The model under review builds one solid part; all positions refer to its coordinate system, in mm. A direction names the side the tool comes from. Round coordinates to 2 decimals unless told otherwise and drop trailing zeros. Order: outer loops, then holes, each group sorted by start corner. A loop starts at its lowest first (then second) coordinate and runs counter-clockwise, first axis right, second up. Notation, with made-up numbers: M 72,26 L 89,26 A21 cw 89,30 Z; hole C -7.75,1 d9. An arc over 180 degrees is marked long. Answer as a JSON object with one key per item and string values. Group by question number.
1. To check wall thickness, follow probe 1 along Z at (x, y) = (-0.5, 9.25); probe 2 along X at (y, z) = (-3.25, 2); probe 3 along X at (y, z) = (-0.5, -55). State the ranges of each line that lie inside material, in increasing order. Write a range as [from, to].
2. Clearance check with flat-ended pins moving along their axes: P1, Ø2, axis at x = -8, z = 170.5, coming from the +Y side; P2, Ø1, axis at y = -7, z = 224.5, coming from the -X side; P3, Ø3, axis at y = 5.5, z = -22.5, coming from the +X side. State where each tip first meets the part, or that it passes through.
3. Machinability: for faces 1 (the face through (4.032, -6.324, -37.264)), 2 (the face through (-5.78, -7.54, 254.46)), 3 (the face through (-1.63, -7.32, 336.24)), which of the approach directions +Z, -Z, +X, -X, +Y, -Y give a long, thin tool a straight path to every point of the face, cutting with its end or side? Answer none if there is none.
4. Add section B-B on z = 219. State the section outline as (x, y) points.
5. Add section A-A on y = 0. State the section outline as (x, z) points, and give its area (3 significant figures).
6. Mouldability with a two-part tool opening along Z and no side actions: class faces 4 (the face through (-9, -4, 253.9)), 5 (the face through (0, 0, -74)), 6 (the face through (-9, -4, 255)), 7 (the face through (-7, 4, 300)) as released by +Z, released by -Z, zero draft, split by the parting line, or undercut.
```python
from build123d import *

# Parameters (mm, degrees)
SKETCH_1_R          = 10
EXTRUDE_1_DEPTH     = 300
SKETCH_2_R          = 6
EXTRUDE_2_DEPTH     = 74
EXTRUDE_START       = 74
SKETCH_3_R          = 6
EXTRUDE_3_DEPTH     = 74
SKETCH_4_R          = 7.5
EXTRUDE_4_DEPTH     = 74
SKETCH_5_R          = 7.5
EXTRUDE_5_DEPTH     = 74
CUT_EXTRUDE_1_DEPTH = 3
CHAMFER_1_SIZE      = 0.5
SKETCH_8_R          = 12.5
SKETCH_8_R_2        = 9.5
CUT_EXTRUDE_2_DEPTH = 1.1


with BuildPart() as part:
    # 草图1 → 凸台-拉伸1 (new body)
    with BuildSketch(Plane.XY):
        with Locations(Location((0, 0, 0), (0, 0, 90))):
            Circle(SKETCH_1_R)
    extrude(amount=EXTRUDE_1_DEPTH)

    # 草图2 → 凸台-拉伸2 (add)
    with BuildSketch(Plane(origin=(0, 0, 0), x_dir=(-1, 0, 0), z_dir=(0, 0, -1))):
        Circle(SKETCH_2_R)
    extrude(amount=EXTRUDE_2_DEPTH)

    # 草图3 → 凸台-拉伸3 (add)
    with BuildSketch(Plane.XY.offset(300).offset(EXTRUDE_START)):
        Circle(SKETCH_3_R)
    extrude(amount=-EXTRUDE_3_DEPTH)

    # 草图4 → 凸台-拉伸4 (add)
    with BuildSketch(Plane.XY.offset(300)):
        Circle(SKETCH_4_R)
    extrude(amount=EXTRUDE_4_DEPTH)

    # 草图5 → 凸台-拉伸5 (add)
    with BuildSketch(Plane(origin=(0, 0, 0), x_dir=(-1, 0, 0), z_dir=(0, 0, -1)).offset(EXTRUDE_START)):
        with Locations(Location((0, 0, 0), (0, 0, 180))):
            Circle(SKETCH_5_R)
    extrude(amount=-EXTRUDE_5_DEPTH)

    # 草图7 → 切除-拉伸1 (cut)
    with BuildSketch(Plane(origin=(0, 7.5, 0), x_dir=(1, 0, 0), z_dir=(0, 1, 0))):
        with BuildLine():
            Line((-2.5, 8), (-2.5, 43))
            ThreePointArc((-2.5, 43), (0, 45.5), (2.5, 43))
            Line((2.5, 43), (2.5, 8))
            ThreePointArc((2.5, 8), (0, 5.5), (-2.5, 8))
        make_face()
        with BuildLine():
            Line((2.5, -308), (2.5, -343))
            ThreePointArc((2.5, -343), (0, -345.5), (-2.5, -343))
            Line((-2.5, -343), (-2.5, -308))
            ThreePointArc((-2.5, -308), (0, -305.5), (2.5, -308))
        make_face()
    extrude(amount=-CUT_EXTRUDE_1_DEPTH, mode=Mode.SUBTRACT)

    # 倒角1
    chamfer_1_edges = [part.edges().sort_by_distance(p)[0] for p in [
        (-7.5, 0, 374),
        (-7.5, 0, -74),
    ]]
    chamfer(chamfer_1_edges, length=CHAMFER_1_SIZE)

    # 草图8 → 切除-拉伸2 (cut)
    with BuildSketch(Plane(origin=(0, 0, 255), x_dir=(-1, 0, 0), z_dir=(0, 0, -1))):
        Circle(SKETCH_8_R)
        with Locations(Location((0, 0, 0), (0, 0, 90))):
            Circle(SKETCH_8_R_2, mode=Mode.SUBTRACT)
    extrude(amount=CUT_EXTRUDE_2_DEPTH, mode=Mode.SUBTRACT)


solid = part.part
```
Recorded:
{
 "1": {"probe 1": "z = [0, 300]", "probe 2": "x = [-9.46, 9.46]", "probe 3": "x = [-7.48, 7.48]"},
 "2": {"P1": "stops at y = 7.14", "P2": "stops at x = -7.6", "P3": "stops at x = 6.34"},
 "3": {"face 1": "-Z", "face 2": "none", "face 3": "+Z"},
 "4": {"outline": "C 0,0 d20"},
 "5": {"outline": "M -10,0 L -7.5,0 L -7.5,-73.5 L -7,-74 L 7,-74 L 7.5,-73.5 L 7.5,0 L 10,0 L 10,253.9 L 9.5,253.9 L 9.5,255 L 10,255 L 10,300 L 7.5,300 L 7.5,373.5 L 7,374 L -7,374 L -7.5,373.5 L -7.5,300 L -10,300 L -10,255 L -9.5,255 L -9.5,253.9 L -10,253.9 Z", "area": "8,220 mm²"},
 "6": {"face 4": "undercut", "face 5": "released by -Z", "face 6": "undercut", "face 7": "released by +Z"}
}
